Source: CAD feature listing. Evaluate the final solid. Frame: model axes, mm. Face numbers are marked on the shaded views. A direction names the side the tool comes from. Give positions to 0.01 mm unless a question says otherwise; leave off trailing zeros. Write each loop counter-clockwise with the first axis right and the second up, starting at its lowest first coordinate (ties: lowest second). Pieces come first, ordered by that corner, then holes. Notation, with made-up numbers: (5, 21.25) -> (46, 21.25) arc R3 ccw to (46, 25.25) -> close; hole circle Ø2 at (64, 2.25). An arc over 180 degrees is marked (long way). Write item = value, one per line.
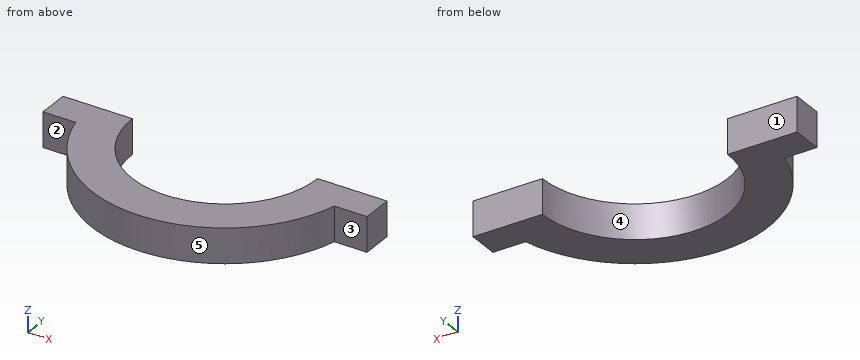
from build123d import *

# Parameters (mm, degrees)
BOSS_EXTRUDE1_DEPTH = 6


with BuildPart() as part:
    # Sketch1 → Boss-Extrude1 (new body)
    with BuildSketch(Plane.XY):
        with BuildLine():
            Line((-16, 50), (-28, 50))
            Line((-28, 50), (-28, 44.637095603))
            Line((-28, 44.637095603), (-22.344508596, 44.637095603))
            ThreePointArc((-22.344508596, 44.637095603), (0, 27.020926738), (22.344508596, 44.637095603))
            Line((22.344508596, 44.637095603), (28, 44.637095603))
            Line((28, 44.637095603), (28, 50))
            Line((28, 50), (16, 50))
            ThreePointArc((16, 50), (0, 34), (-16, 50))
        make_face()
    extrude(amount=BOSS_EXTRUDE1_DEPTH)


solid = part.part
(1) Section query A-A (z = 0.95). Return loops of the section in (x, y).
Values follow:
outline = (-28, 44.64) -> (-22.34, 44.64) arc R22.98 ccw to (22.34, 44.64) -> (28, 44.64) -> (28, 50) -> (16, 50) arc R16 cw to (-16, 50) -> (-28, 50) -> close
(2) First-contact query: pin 1 (1.5 mm diameter, centred on y = 36, z = 1, fed in from -X); pin 2 (1 mm diameter, centred on y = 43.5, z = 2.5, fed in from -X); pin 3 (1.7 mm diameter, centred on x = -26, z = 4.5, fed in from -Y). Flat tips, straight axial feed; report the tip coordinate or a pass-through.
Values follow:
pin_1 = -18.77
pin_2 = -22.18
pin_3 = 44.64
(3) Material intervals for line 1 (X direction, y = 33.5, z = 0.4); line 2 (X direction, y = 35.25, z = 0.6); line 3 (X direction, y = 37.25, z = 1.35), sorted ascending.
Values follow:
line_1 = -15.99 to 15.99
line_2 = -17.62 to -6.2, 6.2 to 17.62
line_3 = -19.12 to -9.67, 9.67 to 19.12
(4) Pull-direction query (X, two-part tool) for the marked faces 3, 4 and 5; classes: pulls with the +X half, pulls with the -X half, needs draft (parallel to the pull), parting line crosses it, or undercut.
Values follow:
face_3 = needs draft
face_4 = undercut
face_5 = parting line crosses it
(5) Access query for the marked faces 1 and 2. Directions: +Z, -Z, +X, -X, +Y, -Y. A direction counts if a zero-diameter tool reaches every point of the face in a straight line with its end or side. Return the directions, or none.
Values follow:
face_1 = +Z, -Z, +X, -X, +Y
face_2 = +Z, -Z, -X, -Y
(6) Section query C-C (x = 0). Return loops of the section in (y, z), plus the area to 3 significant figures.
Values follow:
outline = (27.02, 0) -> (34, 0) -> (34, 6) -> (27.02, 6) -> close
area = 41.9 mm2
(7) Section query B-B (y = 43.25). Return loops of the section in (x, z).
Values follow:
outline = (-21.97, 0) -> (-14.51, 0) -> (-14.51, 6) -> (-21.97, 6) -> close; (14.51, 0) -> (21.97, 0) -> (21.97, 6) -> (14.51, 6) -> close
(8) Section query D-D (y = 37). Return loops of the section in (x, z).
Values follow:
outline = (-18.95, 0) -> (-9.33, 0) -> (-9.33, 6) -> (-18.95, 6) -> close; (9.33, 0) -> (18.95, 0) -> (18.95, 6) -> (9.33, 6) -> close
